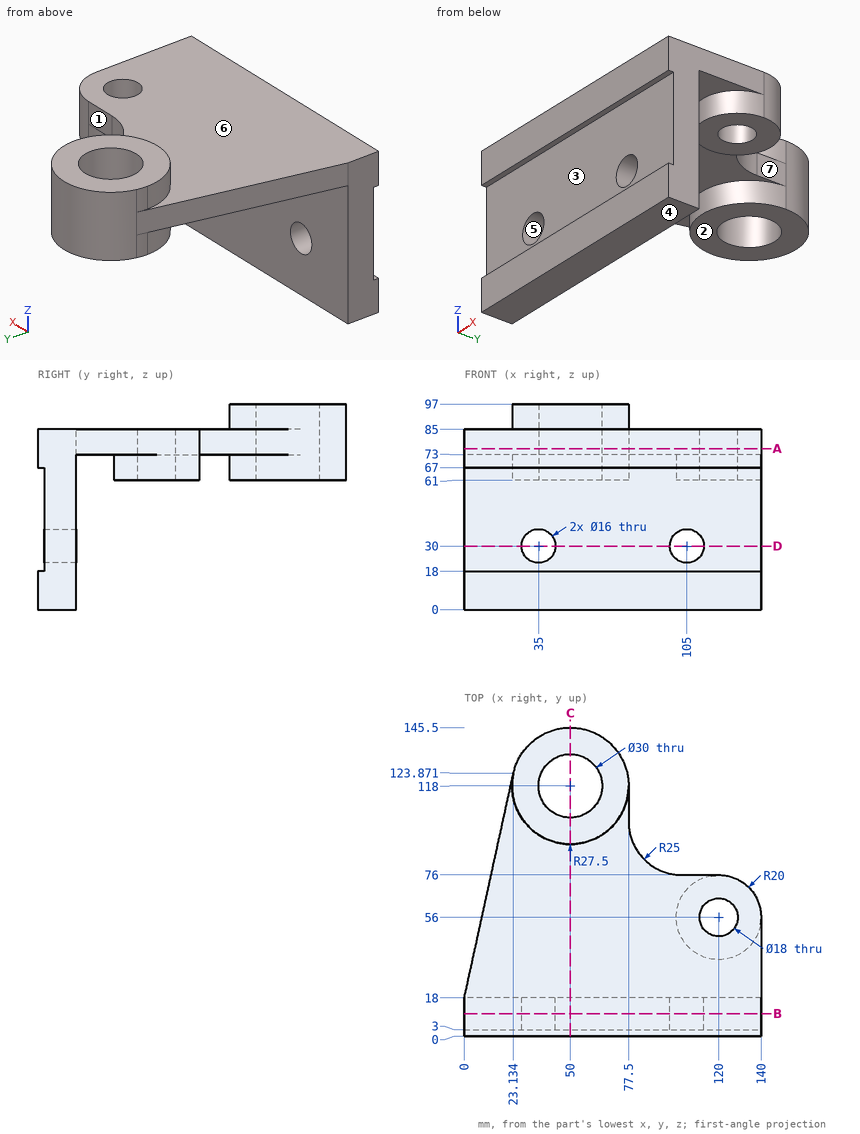
Source: three-view drawing plus pictorial views. Frame: mm from the lowest corner of the part. A direction names the side the tool comes from. Give positions to 0.01 mm unless a question says otherwise; leave off trailing zeros. Write each loop counter-clockwise with the first axis right and the second up, starting at its lowest first coordinate (ties: lowest second). Pieces come first, ordered by that corner, then holes. Notation, with made-up numbers: (69, -7) - (87, -7) arc R16 ccw to (87, 0) - close; hole circle Ø11 at (52.5, -35). An arc over 180 degrees is marked (long way). Write item = value, one per line. Start each with the question number.
1. Section query A-A, the plane z = 76. Output: boundary loops of the cut face in (x, y), then the cut area to 3 significant figures.
2. Ray query, L1, parallel to X at y = 10, z = 30; L2, parallel to Y at x = 46, z = 65.5; L3, parallel to Y at x = 120, z = 75.75. Return the intervals inside material, ascending.
3. Section query B-B, the plane y = 10.5. Output: boundary loops of the cut face in (x, z).
4. First-contact query: pin 1 Ø4 at (x, y) = (55.5, 34.5) entering from -Z; pin 2 Ø20 at (x, y) = (111.5, 64) entering from -Z; pin 3 Ø10 at (x, y) = (117.5, 55) entering from -Z; pin 4 Ø4 at (x, z) = (37, 55) entering from +Y. Flat tips, straight axial feed; report the tip coordinate or a pass-through.
5. Access query for the marked faces 1, 2 and 3. Directions: +Z, -Z, +X, -X, +Y, -Y. A direction counts if a zero-diameter tool reaches every point of the face in a straight line with its end or side. Return the directions, or none.
6. Section query C-C, the plane x = 50. Output: boundary loops of the cut face in (y, z), then the cut area to 3 significant figures.
7. Section query D-D, the plane z = 30. Output: boundary loops of the cut face in (x, y).
8. Mould query, pull axis Z, two halves, no side actions, for the marked faces 4, 5, 6 and 7. Classes: released by +Z, released by -Z, zero draft, split by the parting line, or undercut.
Check sheet entries:
q1.outline = (0, 0) - (140, 0) - (140, 56) arc R20 ccw to (120, 76) - (102.5, 76) arc R25 cw to (77.5, 101) - (77.5, 118) arc R27.5 ccw to (23.13, 123.87) - (0, 18) - close; hole circle Ø30 at (50, 118); hole circle Ø18 at (120, 56)
q1.area = 13,100 mm2
q2.L1 = 0 to 27, 43 to 97, 113 to 140
q2.L2 = 3 to 18, 90.79 to 103.54, 132.46 to 145.21
q2.L3 = 0 to 47, 65 to 76
q3.outline = (0, 0) - (140, 0) - (140, 85) - (0, 85) - close; hole circle Ø16 at (35, 30); hole circle Ø16 at (105, 30)
q4.pin_1 = 73
q4.pin_2 = 61
q4.pin_3 = through
q4.pin_4 = 18
q5.face_1 = +Z, -Z, +X, +Y
q5.face_2 = -Z, +X, -X, +Y
q5.face_3 = +X, -X, -Y
q6.outline = (0, 0) - (18, 0) - (18, 73) - (90.5, 73) - (90.5, 61) - (103, 61) - (103, 97) - (90.5, 97) - (90.5, 85) - (0, 85) - (0, 67) - (3, 67) - (3, 18) - (0, 18) - close; (133, 61) - (145.5, 61) - (145.5, 97) - (133, 97) - close
q6.area = 3,150 mm2
q7.outline = (0, 3) - (27, 3) - (27, 18) - (0, 18) - close; (43, 3) - (97, 3) - (97, 18) - (43, 18) - close; (113, 3) - (140, 3) - (140, 18) - (113, 18) - close
q8.face_4 = released by -Z
q8.face_5 = undercut
q8.face_6 = released by +Z
q8.face_7 = zero draft
